Here's how the part is built. I have some questions about the finished solid (model axes, mm). Give positions to 0.01 mm unless a question says otherwise; leave off trailing zeros. Write each loop counter-clockwise with the first axis right and the second up, starting at its lowest first coordinate (ties: lowest second). Pieces come first, ordered by that corner, then holes. Notation, with made-up numbers: (41.5, -2) -> (64.5, -2) arc R20 ccw to (64.5, 2) -> close; hole circle Ø5 at (81.25, -28.75). An arc over 180 degrees is marked (long way). Use CSV: the item, a comma, the result in double quotes. Start each with the question number.
(1) For pin 1 Ø1 at (x, y) = (1, -12.5) entering from +Z; pin 2 Ø1.5 at (x, z) = (1.5, 14.5) entering from +Y; pin 3 Ø1.9 at (y, z) = (14, 14) entering from +X; pin 4 Ø5 at (y, z) = (14, -14) entering from -X, each with a flat end and sliding along its axis, tell me the tip position at first contact or that it passes through.
(2) I need wall thicknesses on L1, parallel to Z at x = 2.7, y = -13; L2, parallel to Y at x = 1.1, z = 13; L3, parallel to Z at x = 0.25, y = -14. Which ranges of each line are inside material? Lowest first, please. Write a range as [from, to].
(3) Suppose I cut it at C-C on x = 2.3. Give the number of separate pieces and of enclosed holes in the cut face, plus the area to 3 significant figures.
(4) If we mould it in two halves opening along Z, with no side actions, what happens to faces 1 (the cylindrical face through (1.5, 0.1, 19.8)), 2 (the cylindrical face through (1.479, 16.602, -16.702)), 3 (the flat face through (0, 15, -6))? For each: pulls with the +Z half, pulls with the -Z half, needs draft (parallel to the pull), parting line crosses it, or undercut.
(5) Suppose I cut it at A-A on y = 0. List the corners of the cut face in (x, z) for me.
from build123d import *

# Parameters (mm, degrees)
SKETCH_1_R               = 15.75
SKETCH_1_R_2             = 1.6
EXTRUDE_1_DEPTH          = 3
PATTERN_CIRCULAR_1_COUNT = 4
FILLET_1_R               = 2


with BuildPart() as part:
    # 草图1 → 凸台-拉伸1 (new body)
    with BuildSketch(Plane(origin=(0, 0, 0), x_dir=(0, 0, -1), z_dir=(1, 0, 0))):
        with BuildLine():
            ThreePointArc((-16.389345303, 11.109876711), (-19.8, 0), (-16.389345303, -11.109876711))
            ThreePointArc((-16.389345303, -11.109876711), (-16.652364697, -16.652364697), (-11.109876711, -16.389345303))
            ThreePointArc((-11.109876711, -16.389345303), (0, -19.8), (11.109876711, -16.389345303))
            ThreePointArc((11.109876711, -16.389345303), (16.652364697, -16.652364697), (16.389345303, -11.109876711))
            ThreePointArc((16.389345303, -11.109876711), (19.8, 0), (16.389345303, 11.109876711))
            ThreePointArc((16.389345303, 11.109876711), (16.652364697, 16.652364697), (11.109876711, 16.389345303))
            ThreePointArc((11.109876711, 16.389345303), (0, 19.8), (-11.109876711, 16.389345303))
            ThreePointArc((-11.109876711, 16.389345303), (-16.652364697, 16.652364697), (-16.389345303, 11.109876711))
        make_face()
        Circle(SKETCH_1_R, mode=Mode.SUBTRACT)
        with Locations((14.000714267, -14.000714267)):
            Circle(SKETCH_1_R_2, mode=Mode.SUBTRACT)
        with Locations((-14.000714267, -14.000714267)):
            Circle(SKETCH_1_R_2, mode=Mode.SUBTRACT)
        with Locations((-14.000714267, 14.000714267)):
            Circle(SKETCH_1_R_2, mode=Mode.SUBTRACT)
        with Locations((14.000714267, 14.000714267)):
            Circle(SKETCH_1_R_2, mode=Mode.SUBTRACT)
    extrude(amount=EXTRUDE_1_DEPTH)

    # 草图2 → 切除-旋转1 (revolve, cut)
    with BuildSketch(Plane(origin=(0, 0, 0), x_dir=(1, 0, 0), z_dir=(0, -0.7071067811865581, 0.707106781186537)), mode=Mode.PRIVATE) as cut_revolve_1_sk:
        Polygon((0, 19.8), (0, 23.1), (3.3, 19.8), align=None)
    cut_revolve_1 = revolve(cut_revolve_1_sk.sketch.rotate(Axis((3.3, 14.000714267, 14.000714267), (-1, 0, 0)), 315), axis=Axis((3.3, 14.000714267, 14.000714267), (-1, 0, 0)), mode=Mode.SUBTRACT)

    # 阵列(圆周)1: 切除-旋转1 ×4 about axis
    pattern_circular_1_axis = Axis((0, 0, 0), (1, 0, 0))
    for i in range(1, PATTERN_CIRCULAR_1_COUNT):
        add(cut_revolve_1.rotate(pattern_circular_1_axis, i * 360 / PATTERN_CIRCULAR_1_COUNT), mode=Mode.SUBTRACT)

    # 圆角1
    fillet_1_edges = [part.edges().sort_by_distance(p)[0] for p in [
        (1.5, -11.109876711, -16.389345303),
        (1.5, -16.389345303, -11.109876711),
        (1.5, -16.389345303, 11.109876711),
        (1.5, -11.109876711, 16.389345303),
        (1.5, 11.109876711, 16.389345303),
        (1.5, 16.389345303, 11.109876711),
        (1.5, 16.389345303, -11.109876711),
        (1.5, 11.109876711, -16.389345303),
    ]]
    fillet(fillet_1_edges, radius=FILLET_1_R)


solid = part.part
Geometry says:
1,pin 1,"z = 17.61"
1,pin 2,"y = 17.75"
1,pin 3,"through"
1,pin 4,"x = 0.8"
2,L1,"[-17.61, -15.25], [-12.75, -8.89], [8.89, 12.75], [15.25, 17.61]"
2,L2,"[-17.61, -15.96], [-12.04, -8.89], [8.89, 12.04], [15.96, 17.61]"
2,L3,"[-17.75, -17.05], [-10.95, -7.22], [7.22, 10.95], [17.05, 17.75]"
3,separate pieces,"1"
3,enclosed holes,"5"
3,area,"515 mm²"
4,face 1,"pulls with the +Z half"
4,face 2,"undercut"
4,face 3,"needs draft"
5,outline,"(0, -19.8) -> (3, -19.8) -> (3, -15.75) -> (0, -15.75) -> close; (0, 15.75) -> (3, 15.75) -> (3, 19.8) -> (0, 19.8) -> close"
